from build123d import *

# Parameters (mm, degrees)
SKETCH1_R           = 3
SKETCH1_R_2         = 1.5
BOSS_EXTRUDE1_DEPTH = 5


with BuildPart() as part:
    # Sketch1 → Boss-Extrude1 (new body)
    with BuildSketch(Plane.XY):
        Polygon((-20, -10), (-20, 10), (20, 10), (20, -10), (20, -13), (3.5, -13), (3.5, -9.2), (-3.5, -9.2), (-3.5, -13), (-20, -13), align=None)
        Circle(SKETCH1_R, mode=Mode.SUBTRACT)
        with Locations((-17, 7)):
            Circle(SKETCH1_R_2, mode=Mode.SUBTRACT)
        with Locations((17, 7)):
            Circle(SKETCH1_R_2, mode=Mode.SUBTRACT)
    extrude(amount=BOSS_EXTRUDE1_DEPTH)


solid = part.part
Geometry check sheet. Reference: the model listing, model coordinates, mm. A direction names the side the tool comes from. Give positions to 0.01 mm unless a question says otherwise; leave off trailing zeros. Order: outer loops, then holes, each group sorted by start corner. A loop starts at its lowest first (then second) coordinate and runs counter-clockwise, first axis right, second up.
1) Cross-section at B-B (y = 0). Record the boundary of the cut face in (x, z), then the cut area to 3 significant figures.
Results are:
outline: (-20, 0) - (-3, 0) - (-3, 5) - (-20, 5) - close; (3, 0) - (20, 0) - (20, 5) - (3, 5) - close
area: 170 mm2
2) Material ranges on probe 1 along Y at (x, z) = (17, 2.2); probe 2 along Y at (x, z) = (0, 2.3); probe 3 along X at (y, z) = (-10.5, 3.2), recorded low to high.
Results are:
probe 1: y = -13 to 5.5, 8.5 to 10
probe 2: y = -9.2 to -3, 3 to 10
probe 3: x = -20 to -3.5, 3.5 to 20
3) Tool access check on faces 4 (the flat face through (3.5, -11, 2)), 5 (the flat face through (0, 10, 2)). Record the directions out of +Z, -Z, +X, -X, +Y, -Y that give a thin tool (end or side, any length) a straight path to the whole face; none if there is none.
Results are:
face 4: +Z, -Z, -Y
face 5: +Z, -Z, +X, -X, +Y
4) Gauge pin test, flat end, axial feed: pin 1 (1.5 mm diameter, centred on x = -1.5, z = 1.5, fed in from -Y). Record the tip position at first contact, or that the pin passes through.
Results are:
pin 1: stops at y = -9.2
5) Cross-section at A-A (z = 2.05). Record the boundary of the cut face in (x, y), then the cut area to 3 significant figures.
Results are:
outline: (-20, -13) - (-3.5, -13) - (-3.5, -9.2) - (3.5, -9.2) - (3.5, -13) - (20, -13) - (20, 10) - (-20, 10) - close; hole circle Ø3 at (-17, 7); hole circle Ø6 at (0, 0); hole circle Ø3 at (17, 7)
area: 851 mm2
6) Cross-section at C-C (x = 17). Record the boundary of the cut face in (y, z).
Results are:
outline: (-13, 0) - (5.5, 0) - (5.5, 5) - (-13, 5) - close; (8.5, 0) - (10, 0) - (10, 5) - (8.5, 5) - close
7) Draft check along Y on faces 1 (the flat face through (-12, -13, 2)), 2 (the cylindrical face through (15.8, 6.1, 2.5)), 3 (the flat face through (20, -2, 2)). Enter one of: released by +Y, released by -Y, zero draft, split by the parting line, or undercut.
Results are:
face 1: released by -Y
face 2: undercut
face 3: zero draft
8) Cross-section at D-D (y = 8). Record the boundary of the cut face in (x, z), then the cut area to 3 significant figures.
Results are:
outline: (-20, 0) - (-18.12, 0) - (-18.12, 5) - (-20, 5) - close; (-15.88, 0) - (15.88, 0) - (15.88, 5) - (-15.88, 5) - close; (18.12, 0) - (20, 0) - (20, 5) - (18.12, 5) - close
area: 178 mm2
